The figure shows three views and two pictorial views of one solid part (mm, origin at its lowest corner). Answer the questions. A direction names the side the tool comes from. Give positions to 0.01 mm unless a question says otherwise; leave off trailing zeros. Order: outer loops, then holes, each group sorted by start corner. A loop starts at its lowest first (then second) coordinate and runs counter-clockwise, first axis right, second up. Notation, with made-up numbers: (32.5, 8.5) - (75.5, 8.5) arc R28 ccw to (75.5, 43.5) - close; hole circle Ø2 at (-7.75, 24.5). An arc over 180 degrees is marked (long way). Use a Markdown table: item, result. Add a question column.
1. Flat-ended cylindrical pins translate along their axes: P1, Ø6.5, axis at x = 5, z = 5, coming from the -Y side; P2, Ø2, axis at x = 34.5, y = 1.5, coming from the -Z side; P3, Ø2, axis at y = 0.5, z = 13.5, coming from the +X side. Find the tip coordinate at first contact, or state that the pin passes through.
2. A cutting plane is placed at B-B on z = 50. Determine the outline of the cut face in (x, y), and give its area (3 significant figures).
3. Which of the six approach directions +Z, -Z, +X, -X, +Y, -Y give full straight-line access (tool end or side, diameter ignored) to the marked faces 4 and 5?
4. For a pull along X with two mould halves and no side action, classify the marked faces 1, 2 and 3 as released by +X, released by -X, zero draft, split by the parting line, or undercut.
5. Consider L1, parallel to X at y = 2.75, z = 50; L2, parallel to X at y = 3.3, z = 5; L3, parallel to X at y = 2.7, z = 10. Determine where each line is inside the solid, lowest interval first.
6. A cutting plane is placed at D-D on x = 49. Determine the outline of the cut face in (y, z).
7. A cutting plane is placed at C-C on y = 2. Determine the outline of the cut face in (x, z).
8. A cutting plane is placed at A-A on x = 5. Determine the outline of the cut face in (y, z), and give its area (3 significant figures).
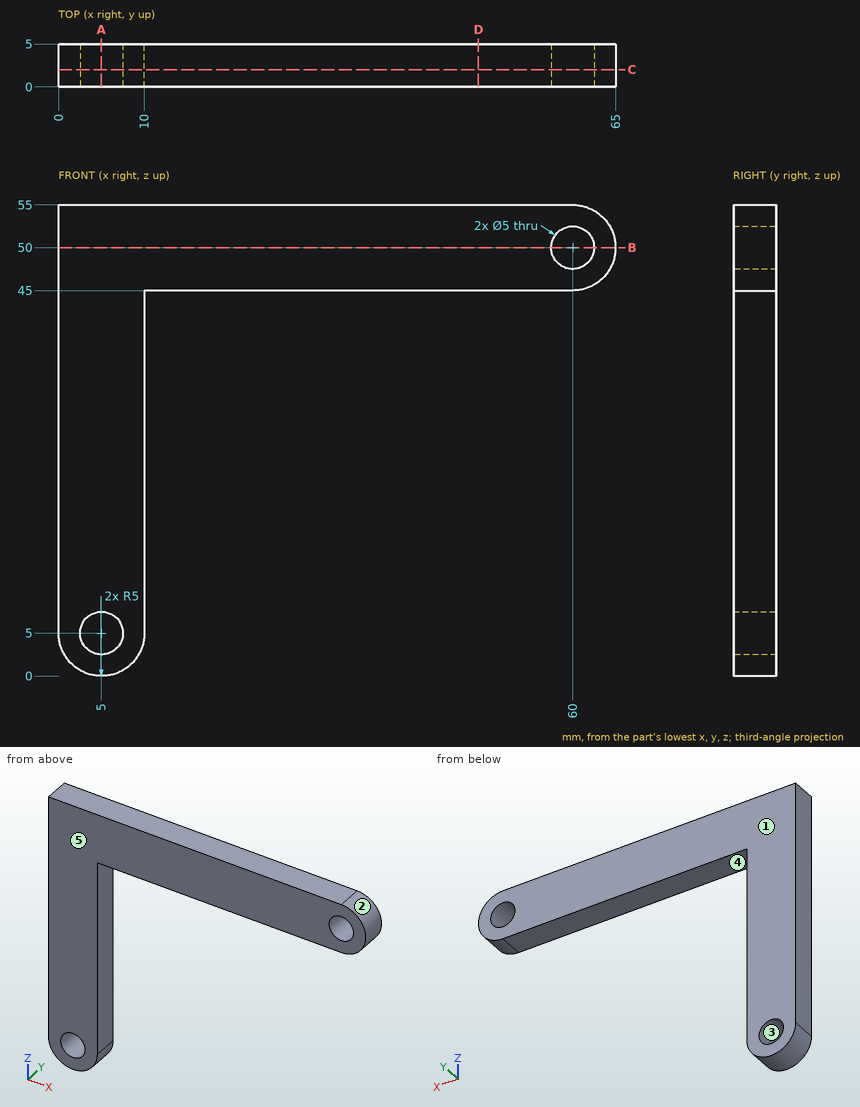
Output values:
| question | item | result |
|---|---|---|
| 1 | P1 | y = 0 |
| 1 | P2 | z = 45 |
| 1 | P3 | x = 10 |
| 2 | outline | (0, 0) - (57.5, 0) - (57.5, 5) - (0, 5) - close; (62.5, 0) - (65, 0) - (65, 5) - (62.5, 5) - close |
| 2 | area | 300 mm² |
| 3 | face 4 | -Z, +X, +Y, -Y |
| 3 | face 5 | +Z, -Z, +X, -X, -Y |
| 4 | face 1 | zero draft |
| 4 | face 2 | released by +X |
| 4 | face 3 | undercut |
| 5 | L1 | 0 to 57.5, 62.5 to 65 |
| 5 | L2 | 0 to 2.5, 7.5 to 10 |
| 5 | L3 | 0 to 10 |
| 6 | outline | (0, 45) - (5, 45) - (5, 55) - (0, 55) - close |
| 7 | outline | (0, 5) arc R5 ccw to (10, 5) - (10, 45) - (60, 45) arc R5 ccw to (60, 55) - (0, 55) - close; hole circle Ø5 at (5, 5); hole circle Ø5 at (60, 50) |
| 8 | outline | (0, 0) - (5, 0) - (5, 2.5) - (0, 2.5) - close; (0, 7.5) - (5, 7.5) - (5, 55) - (0, 55) - close |
| 8 | area | 250 mm² |
